```python
from build123d import *

# Parameters (mm, degrees)
CLAMP_BODY_DEPTH             = 40
PIN_BORE_SKETCH_R            = 14
PIN_BORE_28_DEPTH            = 40
CLAMP_START                  = -40
CLAMP_BORE_64_AND_SLIT_DEPTH = 40
LEVER_START                  = -40
LEVER_ARM_DEPTH              = 40
ARM_WEB_A_DEPTH              = 10
ARM_WEB_B_DEPTH              = 10


with BuildPart() as part:
    # Clamp Body Sketch → Clamp Body (new body)
    with BuildSketch(Plane.XY):
        with BuildLine():
            Line((52, -6), (78.701778719, -6))
            ThreePointArc((78.701778719, -6), (130, 0), (78.701778719, 6))
            Line((78.701778719, 6), (52, 6))
            Line((52, 6), (44.598206242, 6))
            ThreePointArc((44.598206242, 6), (-45, 0), (44.598206242, -6))
            Line((44.598206242, -6), (52, -6))
        make_face()
    extrude(amount=CLAMP_BODY_DEPTH)

    # Pin Bore Sketch → Pin Bore Ø28 (cut)
    with BuildSketch(Plane.XY.offset(40)):
        with Locations((104, 0)):
            Circle(PIN_BORE_SKETCH_R)
    extrude(amount=-PIN_BORE_28_DEPTH, mode=Mode.SUBTRACT)

    # Clamp Bore and Slit Sketch → Clamp Bore Ø64 and Slit (cut)
    with BuildSketch(Plane.XY.offset(40).offset(CLAMP_START)):
        with BuildLine():
            ThreePointArc((-3, -44.899888641), (0, -45), (3, -44.899888641))
            Line((3, -44.899888641), (3, -31.859064644))
            ThreePointArc((3, -31.859064644), (19.483742845, -25.38471518), (30, -11.135528726))
            ThreePointArc((30, -11.135528726), (0, 32), (-30, -11.135528726))
            ThreePointArc((-30, -11.135528726), (-19.483742845, -25.38471518), (-3, -31.859064644))
            Line((-3, -31.859064644), (-3, -44.899888641))
        make_face()
    extrude(amount=CLAMP_BORE_64_AND_SLIT_DEPTH, mode=Mode.SUBTRACT)

    # Lever Arm Sketch → Lever Arm (add)
    with BuildSketch(Plane.XY.offset(40).offset(LEVER_START)):
        with BuildLine():
            Line((-3, -44.899888641), (-3, -74.899888641))
            Line((-3, -74.899888641), (-30, -74.899888641))
            Line((-30, -74.899888641), (-30, -33.541019662))
            ThreePointArc((-30, -33.541019662), (-17.450099602, -41.478838266), (-3, -44.899888641))
        make_face()
        with BuildLine():
            Line((3, -44.899888641), (3, -74.899888641))
            Line((3, -74.899888641), (30, -74.899888641))
            Line((30, -74.899888641), (30, -33.541019662))
            ThreePointArc((30, -33.541019662), (17.450099602, -41.478838266), (3, -44.899888641))
        make_face()
    extrude(amount=LEVER_ARM_DEPTH)

    # Arm Web A Sketch → Arm Web A (add)
    with BuildSketch(Plane(origin=(0, 6, 0), x_dir=(1, 0, 0), z_dir=(0, 1, 0))):
        Polygon((32.912600582, -20), (32.912600582, -17), (88.947224008, -17), (88.947224008, -23), (32.912600582, -23), align=None)
    extrude(amount=ARM_WEB_A_DEPTH)

    # Arm Web B Sketch → Arm Web B (add)
    with BuildSketch(Plane.XZ.offset(6)):
        Polygon((44.598206242, 23), (37.493332774, 23), (37.493332774, 20), (86.340481081, 20), (86.340481081, 23), align=None)
    extrude(amount=ARM_WEB_B_DEPTH)


solid = part.part
```
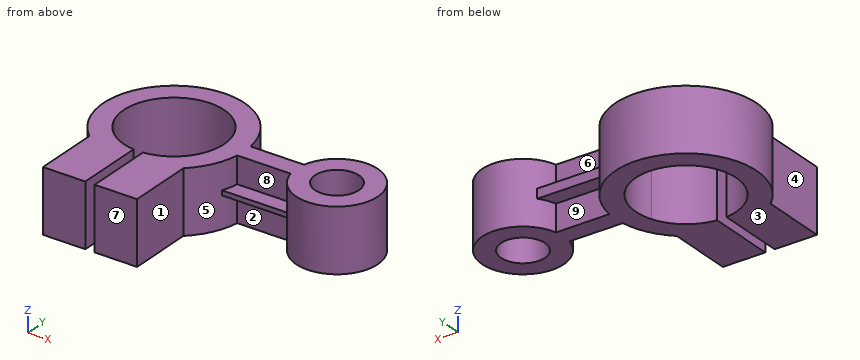
Input: part model. Units: mm. Frame: model coordinates. Face numbers are marked on the shaded views. A direction names the side the tool comes from. Round coordinates to 2 decimals unless told otherwise and drop trailing zeros. Write each loop counter-clockwise with the first axis right and the second up, starting at its lowest first coordinate (ties: lowest second). Pieces come first, ordered by that corner, then holes. Notation, with made-up numbers: (-10.5, 19.25) - (3.5, 19.25) arc R19 ccw to (3.5, 26.25) - close; hole circle Ø10 at (65.5, 34.25). An arc over 180 degrees is marked (long way). Write item = value, one per line.
(1) Section query A-A on y = 0. Output: boundary loops of the cut face in (x, z).
Geometry check:
outline = (-45, 0) - (-32, 0) - (-32, 40) - (-45, 40) - close; (32, 0) - (90, 0) - (90, 40) - (32, 40) - close; (118, 0) - (130, 0) - (130, 40) - (118, 40) - close
(2) Section query C-C on z = 13.5. Output: boundary loops of the cut face in (x, y).
Geometry check:
outline = (-30, -74.9) - (-3, -74.9) - (-3, -31.86) arc R32 cw (long way) to (3, -31.86) - (3, -74.9) - (30, -74.9) - (30, -33.54) arc R45 ccw to (44.6, -6) - (78.7, -6) arc R26 ccw (long way) to (78.7, 6) - (44.6, 6) arc R45 ccw (long way) to (-30, -33.54) - close; hole circle Ø28 at (104, 0)
(3) Section query B-B on x = 104. Output: boundary loops of the cut face in (y, z), then the cut area to 3 significant figures.
Geometry check:
outline = (-26, 0) - (-14, 0) - (-14, 40) - (-26, 40) - close; (14, 0) - (26, 0) - (26, 40) - (14, 40) - close
area = 960 mm^2
(4) Section query D-D on y = -62.5. Output: boundary loops of the cut face in (x, z).
Geometry check:
outline = (-30, 0) - (-3, 0) - (-3, 40) - (-30, 40) - close; (3, 0) - (30, 0) - (30, 40) - (3, 40) - close
(5) Material intervals for probe 1 along Y at (x, z) = (104, 29); probe 2 along X at (y, z) = (-49, 20); probe 3 along X at (y, z) = (-8, 37), sorted ascending.
Geometry check:
probe_1 = -26 to -14, 14 to 26
probe_2 = -30 to -3, 3 to 30
probe_3 = -44.28 to -30.98, 30.98 to 44.28, 79.26 to 92.51, 115.49 to 128.74
(6) Access query for the marked faces 5, 6, 7, 8 and 9. Directions: +Z, -Z, +X, -X, +Y, -Y. A direction counts if a zero-diameter tool reaches every point of the face in a straight line with its end or side. Return the directions, or none.
Geometry check:
face_5 = -Y
face_6 = +Z, +Y
face_7 = +Z, -Z, +X, -X, -Y
face_8 = +Z, -Y
face_9 = -Z, +Y
(7) Pull-direction query (X, two-part tool) for the marked faces 1, 2, 3 and 4; classes: +X half, -X half, draft (parallel to the pull), parting line (faces both ways), or undercut.
Geometry check:
face_1 = +X half
face_2 = undercut
face_3 = draft
face_4 = -X half
(8) Contact query for flat-ended pins moving along their axis: pin 1 Ø5 at (x, z) = (70, 27.5) entering from +Y; pin 2 Ø0.9 at (x, z) = (60, 22) entering from -Y; pin 3 Ø8 at (x, y) = (71.5, -12.5) entering from +Z. Output: stop coordinate, or through.
Geometry check:
pin_1 = 6
pin_2 = -16
pin_3 = 23
